from build123d import *

# Parameters (mm, degrees)
SKETCH1_W           = 45
SKETCH1_H           = 64
BOSS_EXTRUDE1_DEPTH = 5
SKETCH_2_3_W        = 18
SKETCH_2_3_H        = 30
CUT_EXTRUDE1_DEPTH  = 40.436658073
CUT_EXTRUDE2_DEPTH  = 3
FILLET1_R           = 3


with BuildPart() as part:
    # Sketch1 → Boss-Extrude1 (new body)
    with BuildSketch(Plane(origin=(0, 0, 0), x_dir=(1, 0, 0), z_dir=(0, 1, 0))):
        Rectangle(SKETCH1_W, SKETCH1_H)
    extrude(amount=BOSS_EXTRUDE1_DEPTH)

    # Sketch 2_3 → Cut-Extrude1 (cut, through all)
    with BuildSketch(Plane(origin=(0, 5, 0), x_dir=(1, 0, 0), z_dir=(0, 1, 0))):
        Rectangle(SKETCH_2_3_W, SKETCH_2_3_H)
        with BuildLine():
            Line((-9, -22.7), (9, -22.7))
            ThreePointArc((9, -22.7), (11.15, -24.85), (9, -27))
            Line((9, -27), (-9, -27))
            ThreePointArc((-9, -27), (-11.15, -24.85), (-9, -22.7))
        make_face()
        with BuildLine():
            Line((-9, 22.7), (9, 22.7))
            ThreePointArc((9, 22.7), (11.15, 24.85), (9, 27))
            Line((9, 27), (-9, 27))
            ThreePointArc((-9, 27), (-11.15, 24.85), (-9, 22.7))
        make_face()
    extrude(amount=-CUT_EXTRUDE1_DEPTH, mode=Mode.SUBTRACT)

    # Sketch 2_3 2 → Cut-Extrude2 (cut)
    with BuildSketch(Plane(origin=(0, 5, 0), x_dir=(1, 0, 0), z_dir=(0, 1, 0))):
        with BuildLine():
            Line((-9, -20.7), (9, -20.7))
            ThreePointArc((9, -20.7), (13.15, -24.85), (9, -29))
            Line((9, -29), (-9, -29))
            ThreePointArc((-9, -29), (-13.15, -24.85), (-9, -20.7))
        make_face()
        with BuildLine():
            Line((-9, 20.7), (9, 20.7))
            ThreePointArc((9, 20.7), (13.15, 24.85), (9, 29))
            Line((9, 29), (-9, 29))
            ThreePointArc((-9, 29), (-13.15, 24.85), (-9, 20.7))
        make_face()
    extrude(amount=-CUT_EXTRUDE2_DEPTH, mode=Mode.SUBTRACT)

    # Fillet1
    fillet1_edges = [part.edges().sort_by_distance(p)[0] for p in [
        (-9, 2.5, -15),
        (9, 2.5, -15),
        (9, 2.5, 15),
        (-9, 2.5, 15),
    ]]
    fillet(fillet1_edges, radius=FILLET1_R)


solid = part.part
Work out the finished part from the listing and answer in its coordinate system (mm). A direction names the side the tool comes from. Round coordinates to 2 decimals unless told otherwise and drop trailing zeros. Write each loop counter-clockwise with the first axis right and the second up, starting at its lowest first coordinate (ties: lowest second). Pieces come first, ordered by that corner, then holes. Notation, with made-up numbers: (-9.75, 69.5) -> (3.25, 69.5) arc R9 cw to (3.25, 75.5) -> close; hole circle Ø6 at (5, -6.5). An arc over 180 degrees is marked (long way). Write each question's results on one line, items separated by ' | '.
Item 1: A cutting plane is placed at C-C, the plane x = 1. Determine the outline of the cut face in (y, z).
Result set:
outline: (0, -32) -> (5, -32) -> (5, -29) -> (2, -29) -> (2, -27) -> (0, -27) -> close; (0, -22.7) -> (2, -22.7) -> (2, -20.7) -> (5, -20.7) -> (5, -15) -> (0, -15) -> close; (0, 15) -> (5, 15) -> (5, 20.7) -> (2, 20.7) -> (2, 22.7) -> (0, 22.7) -> close; (0, 27) -> (2, 27) -> (2, 29) -> (5, 29) -> (5, 32) -> (0, 32) -> close
Item 2: Find the intervals of material crossed by line 1 along Z through (x, y) = (-1.5, 1.2); line 2 along Z through (x, y) = (1.5, 2.95); line 3 along X through (y, z) = (1.3, -8), in increasing order. Write a range as [from, to].
Result set:
line 1: [-32, -27], [-22.7, -15], [15, 22.7], [27, 32] | line 2: [-32, -29], [-20.7, -15], [15, 20.7], [29, 32] | line 3: [-22.5, -9], [9, 22.5]
Item 3: The mould has two halves that part along Z. Classify faces 1 (the face through (-9, 3, 0)), 2 (the face through (-22.5, 2, 0)), 3 (the face through (13.15, 3.52, -24.76)), 4 (the face through (0, 2, -32)): +Z half, -Z half, draft (parallel to the pull), parting line (faces both ways), or undercut.
Result set:
face 1: undercut | face 2: draft | face 3: undercut | face 4: -Z half
Item 4: Flat-ended cylindrical pins translate along their axes: P1, Ø9, axis at x = 0.5, z = 24.5, coming from the +Y side; P2, Ø6.5, axis at x = 0.5, z = -24, coming from the +Y side. Find the tip coordinate at first contact, or state that the pin passes through.
Result set:
P1: y = 5 | P2: y = 2
Item 5: A cutting plane is placed at D-D, the plane z = 24.85. Determine the outline of the cut face in (x, y), plus the area to 4 significant figures.
Result set:
outline: (-22.5, 0) -> (-11.15, 0) -> (-11.15, 2) -> (-13.15, 2) -> (-13.15, 5) -> (-22.5, 5) -> close; (11.15, 0) -> (22.5, 0) -> (22.5, 5) -> (13.15, 5) -> (13.15, 2) -> (11.15, 2) -> close | area: 101.5 mm^2
Item 6: A cutting plane is placed at A-A, the plane z = 10.5. Determine the outline of the cut face in (x, y).
Result set:
outline: (-22.5, 0) -> (-9, 0) -> (-9, 5) -> (-22.5, 5) -> close; (9, 0) -> (22.5, 0) -> (22.5, 5) -> (9, 5) -> close
Item 7: A cutting plane is placed at B-B, the plane y = 2.75. Determine the outline of the cut face in (x, z).
Result set:
outline: (-22.5, -32) -> (22.5, -32) -> (22.5, 32) -> (-22.5, 32) -> close; hole (-9, -29) -> (9, -29) arc R4.15 ccw to (9, -20.7) -> (-9, -20.7) arc R4.15 ccw to start; hole (-9, -12) arc R3 ccw to (-6, -15) -> (6, -15) arc R3 ccw to (9, -12) -> (9, 12) arc R3 ccw to (6, 15) -> (-6, 15) arc R3 ccw to (-9, 12) -> close; hole (-9, 20.7) -> (9, 20.7) arc R4.15 ccw to (9, 29) -> (-9, 29) arc R4.15 ccw to start
Item 8: Which of the six approach directions +Z, -Z, +X, -X, +Y, -Y give full straight-line access (tool end or side, diameter ignored) to faces 5 (the face through (0, 4, -20.7)), 6 (the face through (-10, 5, 0)), 7 (the face through (0, 1, -22.7))?
Result set:
face 5: +Y | face 6: +Z, -Z, +X, -X, +Y | face 7: +Y, -Y
